Here's how the part is built. I have some questions about the finished solid (model axes, mm). Round coordinates to 2 decimals unless told otherwise and drop trailing zeros. Write each loop counter-clockwise with the first axis right and the second up, starting at its lowest first coordinate (ties: lowest second). Pieces come first, ordered by that corner, then holes. Notation, with made-up numbers: M -13,-13 L 10,-13 A19 ccw 10,3 Z; hole C 68.25,31 d1. An arc over 180 degrees is marked long. Use a Markdown table: item, result. Add a question column.
```python
from build123d import *

# Parameters (mm, degrees)
SKETCH1_W           = 30
SKETCH1_H           = 10
BOSS_EXTRUDE1_DEPTH = 5
SKETCH2_R           = 2.25
CUT_EXTRUDE1_DEPTH  = 10


with BuildPart() as part:
    # Sketch1 → Boss-Extrude1 (new body)
    with BuildSketch(Plane(origin=(0, 0, 0), x_dir=(1, 0, 0), z_dir=(0, 1, 0))):
        Rectangle(SKETCH1_W, SKETCH1_H)
    extrude(amount=BOSS_EXTRUDE1_DEPTH)

    # Sketch2 → Cut-Extrude1 (cut)
    with BuildSketch(Plane(origin=(0, 5, 0), x_dir=(1, 0, 0), z_dir=(0, 1, 0))):
        with Locations(Location((-11, 0, 0), (0, 0, 270))):
            Circle(SKETCH2_R)
        with Locations(Location((11, 0, 0), (0, 0, 270))):
            Circle(SKETCH2_R)
    extrude(amount=-CUT_EXTRUDE1_DEPTH, mode=Mode.SUBTRACT)


solid = part.part
```
Item 1: Imagine slicing it at C-C on y = 4. List the corners of the cut face in (x, z) for me, plus the area to 3 significant figures.
Item 2: I need wall thicknesses on probe 1 along X at (y, z) = (3.55, 0); probe 2 along X at (y, z) = (2.45, 1.75); probe 3 along Z at (x, y) = (-9, 4.6). Which ranges of each line are inside material? Lowest first, please. Write a range as from..to.
Item 3: Imagine slicing it at B-B on z = 0. List the corners of the cut face in (x, y) for me.
Item 4: Imagine slicing it at A-A on x = 11. List the corners of the cut face in (y, z) for me.
Item 5: For pin 1 Ø3.5 at (x, z) = (11, 0) entering from +Y, with a flat end and sliding along its axis, tell me the tip position at first contact or that it passes through.
The answers:
| question | item | result |
|---|---|---|
| 1 | outline | M -15,-5 L 15,-5 L 15,5 L -15,5 Z; hole C -11,0 d4.5; hole C 11,0 d4.5 |
| 1 | area | 268 mm² |
| 2 | probe 1 | -15..-13.25, -8.75..8.75, 13.25..15 |
| 2 | probe 2 | -15..-12.41, -9.59..9.59, 12.41..15 |
| 2 | probe 3 | -5..-1.03, 1.03..5 |
| 3 | outline | M -15,0 L -13.25,0 L -13.25,5 L -15,5 Z; M -8.75,0 L 8.75,0 L 8.75,5 L -8.75,5 Z; M 13.25,0 L 15,0 L 15,5 L 13.25,5 Z |
| 4 | outline | M 0,-5 L 5,-5 L 5,-2.25 L 0,-2.25 Z; M 0,2.25 L 5,2.25 L 5,5 L 0,5 Z |
| 5 | pin 1 | through |
